The drawing under review shows one solid part. Ordinate dimensions are in mm from its lowest x, y, z. A direction names the side the tool comes from. Coordinates: 2 decimals unless noted, no trailing zeros. Order: outer loops, then holes, each group sorted by start corner. A loop starts at its lowest first (then second) coordinate and runs counter-clockwise, first axis right, second up. Notation, with made-up numbers: M 82,26 L 97,26 A25 cw 97,59 Z; hole C 10.5,-17 d2. An arc over 180 degrees is marked long. Answer as a JSON object with one key per item and string values.
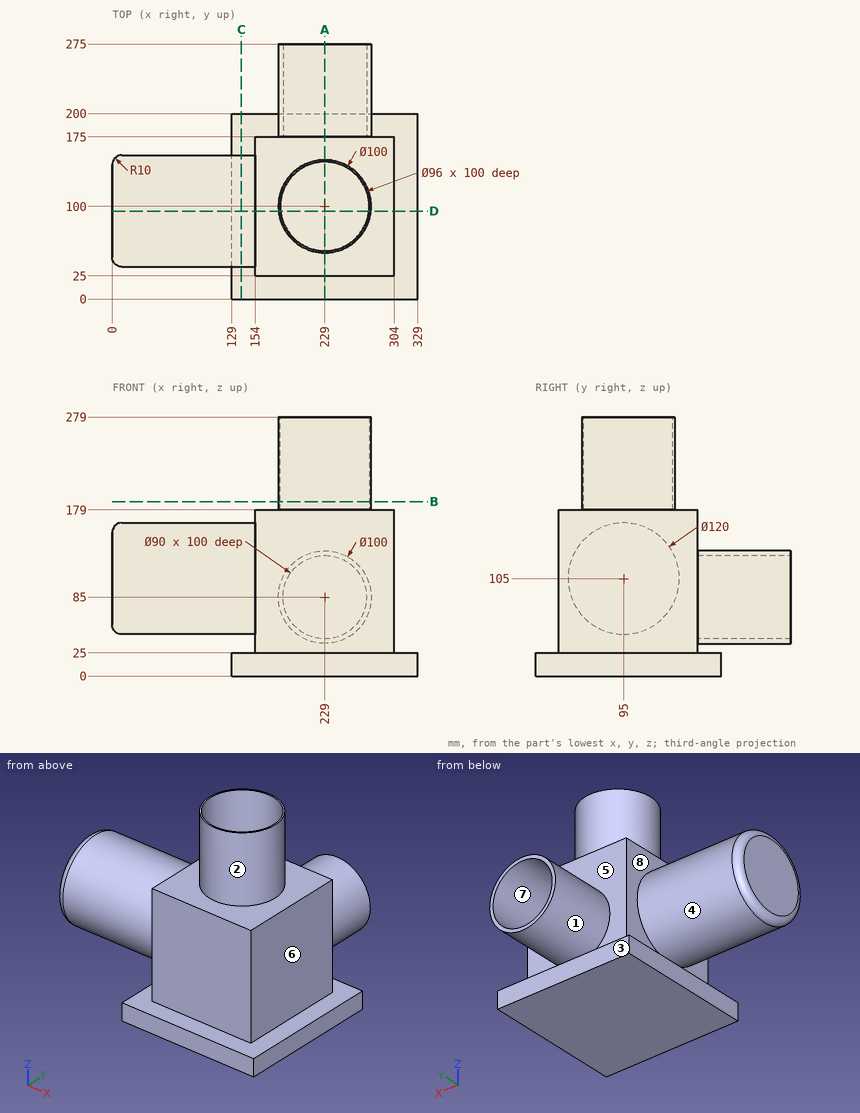
1) To check wall thickness, follow L1, parallel to Z at x = 256.5, y = 197.5; L2, parallel to X at y = 232, z = 85; L3, parallel to Y at x = 232, z = 185.5. State the ranges of each line that lie inside material, in increasing order.
Taken from the geometry:
{"L1": "z = 0 to 25, 43.24 to 49.38, 120.62 to 126.76", "L2": "x = 179 to 184, 274 to 279", "L3": "y = 50.09 to 52.09, 147.91 to 149.91"}
2) Tool access review of the marked faces 1, 2, 3 and 4: name each direction out of +Z, -Z, +X, -X, +Y, -Y from which nothing blocks a thin tool from reaching the whole face with its end or side.
Taken from the geometry:
{"face 1": "+Y", "face 2": "+Z", "face 3": "-Z, +X, -X, +Y", "face 4": "-X"}
3) Add section C-C (x = 139). State the section outline as (y, z) points.
Taken from the geometry:
{"outline": "M 0,0 L 200,0 L 200,25 L 0,25 Z; C 95,105 d120"}
4) Add section D-D (y = 95). State the section outline as (x, z) points.
Taken from the geometry:
{"outline": "M 0,55 A10 ccw 10,45 L 154,45 L 154,25 L 129,25 L 129,0 L 329,0 L 329,25 L 304,25 L 304,179 L 278.75,179 L 278.75,279 L 276.74,279 L 276.74,179 L 181.26,179 L 181.26,279 L 179.25,279 L 179.25,179 L 154,179 L 154,165 L 10,165 A10 ccw 0,155 Z"}
5) Insertion check: pin 1 Ø1.5 at (x, y) = (189, 231) entering from +Z; pin 2 Ø7.5 at (x, z) = (213.5, 9.5) entering from +Y; pin 3 Ø4 at (y, z) = (223.5, 49) entering from -X. Each pin has a flat end and moves straight along its axis. Give the tip position at first contact, or say it passes through.
Taken from the geometry:
{"pin 1": "stops at z = 115.97", "pin 2": "stops at y = 200", "pin 3": "stops at x = 192.34"}
6) Mouldability with a two-part tool opening along X and no side actions: class the marked faces 5, 6, 7 and 8 as released by +X, released by -X, zero draft, split by the parting line, or undercut.
Taken from the geometry:
{"face 5": "zero draft", "face 6": "released by +X", "face 7": "undercut", "face 8": "released by -X"}
7) Add section A-A (x = 229). State the section outline as (y, z) points.
Taken from the geometry:
{"outline": "M 0,0 L 200,0 L 200,25 L 175,25 L 175,35 L 275,35 L 275,40 L 175,40 L 175,130 L 275,130 L 275,135 L 175,135 L 175,179 L 150,179 L 150,279 L 148,279 L 148,179 L 52,179 L 52,279 L 50,279 L 50,179 L 25,179 L 25,25 L 0,25 Z"}
8) Add section B-B (z = 188). State the section outline as (x, y) points, and give its area (3 significant figures).
Taken from the geometry:
{"outline": "C 229,100 d100; hole C 229,100 d96", "area": "616 mm2"}
